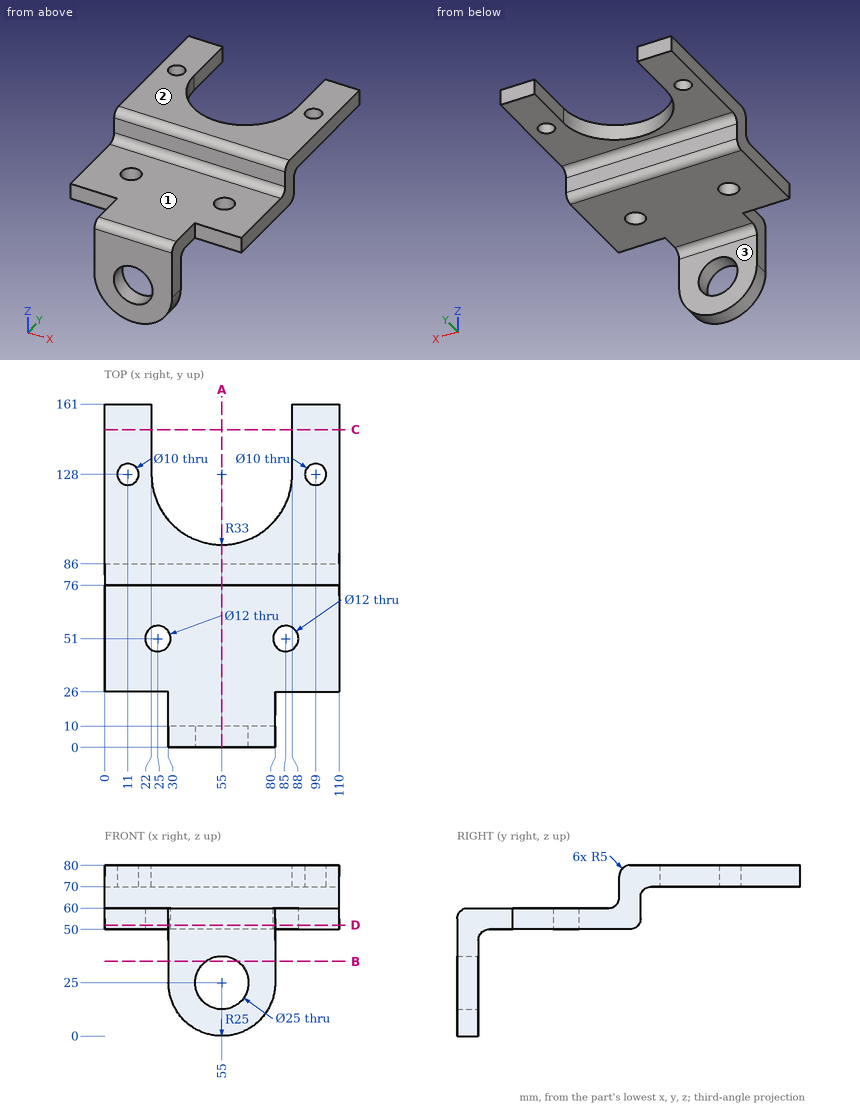
The drawing under review shows one solid part. Ordinate dimensions are in mm from its lowest x, y, z. A direction names the side the tool comes from. Give positions to 0.01 mm unless a question says otherwise; leave off trailing zeros. Order: outer loops, then holes, each group sorted by start corner. A loop starts at its lowest first (then second) coordinate and runs counter-clockwise, first axis right, second up. Notation, with made-up numbers: (40.5, 39.25) - (76.5, 39.25) arc R22 ccw to (76.5, 65.25) - close; hole circle Ø5 at (16, 51.5). An arc over 180 degrees is marked (long way). Answer as a JSON object with one key per item and string values. Group by question number.
Item 1: Take a section at D-D on z = 52. Give the boundary of the cut face in (x, y), and give its area (3 significant figures).
Item 2: Machinability: for the marked faces 1, 2 and 3, which of the approach directions +Z, -Z, +X, -X, +Y, -Y give a long, thin tool a straight path to every point of the face, cutting with its end or side? Answer none if there is none.
Item 3: Take a section at A-A on x = 55. Give the boundary of the cut face in (y, z).
Item 4: Take a section at B-B on z = 35. Give the boundary of the cut face in (x, y).
Item 5: Clearance check with flat-ended pins moving along their axes: pin 1 Ø20 at (x, y) = (65.5, 43.5) entering from +Z; pin 2 Ø8 at (x, y) = (99, 128) entering from +Z; pin 3 Ø16 at (x, y) = (11, 128) entering from +Z; pin 4 Ø5 at (x, z) = (71.5, 59.5) entering from +Y. State where each tip first meets the part, or that it passes through.
Item 6: Take a section at C-C on y = 149. Give the boundary of the cut face in (x, z), and give its area (3 significant figures).
Item 7: Wall thickness on line 1 along Y through (x, z) = (85, 55); line 2 along Y through (x, z) = (54, 65); line 3 along Z through (x, y) = (16, 131): over which ranges is each line inside the solid? List them lowest first.
Reported:
{
 "1": {"outline": "(0, 26) - (30, 26) - (30, 0) - (80, 0) - (80, 26) - (110, 26) - (110, 85) - (0, 85) - close; hole circle Ø12 at (25, 51); hole circle Ø12 at (85, 51)", "area": "7,560 mm^2"},
 "2": {"face 1": "+Z, +X, -X, -Y", "face 2": "+Z, +X, -X, +Y, -Y", "face 3": "-Z, +X, -X, +Y"},
 "3": {"outline": "(0, 0) - (10, 0) - (10, 12.5) - (0, 12.5) - close; (0, 37.5) - (10, 37.5) - (10, 45) arc R5 cw to (15, 50) - (81, 50) arc R5 ccw to (86, 55) - (86, 65) arc R5 cw to (91, 70) - (95, 70) - (95, 80) - (81, 80) arc R5 ccw to (76, 75) - (76, 65) arc R5 cw to (71, 60) - (5, 60) arc R5 ccw to (0, 55) - close"},
 "4": {"outline": "(30, 0) - (47.5, 0) - (47.5, 10) - (30, 10) - close; (62.5, 0) - (80, 0) - (80, 10) - (62.5, 10) - close"},
 "5": {"pin 1": "z = 60", "pin 2": "through", "pin 3": "z = 80", "pin 4": "y = 86"},
 "6": {"outline": "(0, 70) - (22, 70) - (22, 80) - (0, 80) - close; (88, 70) - (110, 70) - (110, 80) - (88, 80) - close", "area": "440 mm^2"},
 "7": {"line 1": "26 to 45, 57 to 86", "line 2": "76 to 86", "line 3": "70 to 80"}
}
